from build123d import *

# Parameters (mm, degrees)
NUT_BODY_7MM_DEPTH      = 3.5
BORE_15_DEPTH           = 21.137030566
BORE_15_DEPTH_BACK      = 21.137030566
BORE_SKETCH_15_R        = 7.5
EDGE_CHAMFERS_1X45_SIZE = 1


with BuildPart() as part:
    # Slotted Nut Profile Ø27 → Nut Body 7mm (new, symmetric)
    with BuildSketch(Plane.XY):
        with BuildLine():
            Line((2, 11.351029923), (2, 13.351029923))
            ThreePointArc((2, 13.351029923), (9.545941546, 9.545941546), (13.351029923, 2))
            Line((13.351029923, 2), (11.351029923, 2))
            Line((11.351029923, 2), (11.351029923, -2))
            Line((11.351029923, -2), (13.351029923, -2))
            ThreePointArc((13.351029923, -2), (9.545941546, -9.545941546), (2, -13.351029923))
            Line((2, -13.351029923), (2, -11.351029923))
            Line((2, -11.351029923), (-2, -11.351029923))
            Line((-2, -11.351029923), (-2, -13.351029923))
            ThreePointArc((-2, -13.351029923), (-9.545941546, -9.545941546), (-13.351029923, -2))
            Line((-13.351029923, -2), (-11.351029923, -2))
            Line((-11.351029923, -2), (-11.351029923, 2))
            Line((-11.351029923, 2), (-13.351029923, 2))
            ThreePointArc((-13.351029923, 2), (-9.545941546, 9.545941546), (-2, 13.351029923))
            Line((-2, 13.351029923), (-2, 11.351029923))
            Line((-2, 11.351029923), (2, 11.351029923))
        make_face()
    extrude(amount=NUT_BODY_7MM_DEPTH, both=True)

    # Bore Sketch Ø15 → Bore Ø15 (cut, two sides: drawn at the far end of the back side and taken through both)
    with BuildSketch(Plane.XY.offset(3.5).offset(-BORE_15_DEPTH_BACK)):
        Circle(BORE_SKETCH_15_R)
    extrude(amount=BORE_15_DEPTH + BORE_15_DEPTH_BACK, mode=Mode.SUBTRACT)

    # Edge Chamfers 1x45°
    edge_chamfers_1x45_edges = [part.edges().sort_by_distance(p)[0] for p in [
        (-9.545941546, 9.545941546, 3.5),
        (-9.545941546, -9.545941546, 3.5),
        (9.545941546, -9.545941546, 3.5),
        (9.545941546, 9.545941546, 3.5),
    ]]
    chamfer(edge_chamfers_1x45_edges, length=EDGE_CHAMFERS_1X45_SIZE)


solid = part.part
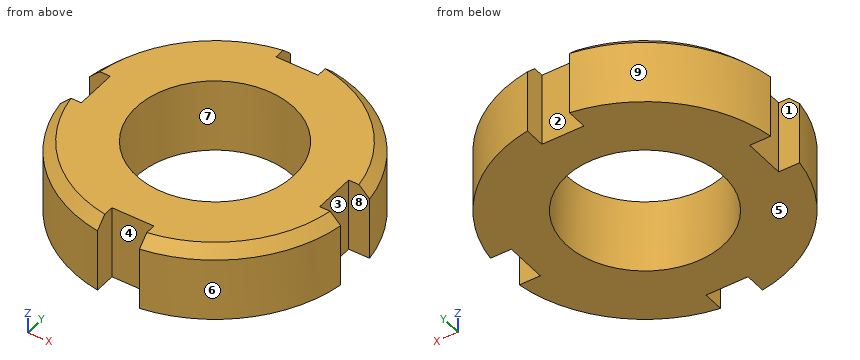
Design review of the part built by this model. Coordinates are the model's own, in mm. Face numbers are marked on the shaded views. A direction names the side the tool comes from. Round coordinates to 2 decimals unless told otherwise and drop trailing zeros. Write each loop counter-clockwise with the first axis right and the second up, starting at its lowest first coordinate (ties: lowest second). Pieces come first, ordered by that corner, then holes. Notation, with made-up numbers: (-22, 14) - (-12, 14) arc R27 ccw to (-12, 49) - close; hole circle Ø2 at (59, 39). An arc over 180 degrees is marked (long way). Use a Markdown table: item, result. Add a question column.
1. We need section C-C (z = -3). State the section outline as (x, y) points.
2. Clearance check with flat-ended pins moving along their axes: pin 1 (1.2 mm diameter, centred on x = 0, z = -1, fed in from +Y); pin 2 (2 mm diameter, centred on y = 0.5, z = 1.5, fed in from +X); pin 3 (1 mm diameter, centred on y = -12, z = -1, fed in from +X). State where each tip first meets the part, or that it passes through.
3. We need section A-A (x = 0). State the section outline as (y, z) points.
4. Mouldability with a two-part tool opening along Y and no side actions: class the marked faces 6, 7, 8 and 9 as +Y half, -Y half, draft (parallel to the pull), parting line (faces both ways), or undercut.
5. For the marked faces 1, 2, 3, 4 and 5, list the 3-axis set-ups (+Z, -Z, +X, -X, +Y, -Y) from which the entire face can be reached by the end or side of a thin tool; tool diameter is ignored.
6. Wall thickness on probe 1 along X at (y, z) = (0, 1); probe 2 along X at (y, z) = (-2.5, 3.25): over which ranges is each line inside the solid? List them lowest first.
Output:
| question | item | result |
|---|---|---|
| 1 | outline | (-13.35, -2) arc R13.5 ccw to (-2, -13.35) - (-2, -11.35) - (2, -11.35) - (2, -13.35) arc R13.5 ccw to (13.35, -2) - (11.35, -2) - (11.35, 2) - (13.35, 2) arc R13.5 ccw to (2, 13.35) - (2, 11.35) - (-2, 11.35) - (-2, 13.35) arc R13.5 ccw to (-13.35, 2) - (-11.35, 2) - (-11.35, -2) - close; hole circle Ø15 at (0, 0) |
| 2 | pin 1 | stops at y = 11.35 |
| 2 | pin 2 | stops at x = 11.35 |
| 2 | pin 3 | stops at x = 7.07 |
| 3 | outline | (-11.35, -3.5) - (-7.5, -3.5) - (-7.5, 3.5) - (-11.35, 3.5) - close; (7.5, -3.5) - (11.35, -3.5) - (11.35, 3.5) - (7.5, 3.5) - close |
| 4 | face 6 | -Y half |
| 4 | face 7 | undercut |
| 4 | face 8 | undercut |
| 4 | face 9 | +Y half |
| 5 | face 1 | +Z, -Z, -X |
| 5 | face 2 | +Z, -Z, +Y |
| 5 | face 3 | +Z, -Z, +X |
| 5 | face 4 | +Z, -Z, -Y |
| 5 | face 5 | -Z, +X, -X, +Y, -Y |
| 6 | probe 1 | x = -11.35 to -7.5, 7.5 to 11.35 |
| 6 | probe 2 | x = -12.5 to -7.07, 7.07 to 12.5 |
